The model under review builds one solid part; all positions refer to its coordinate system, in mm. Face numbers are marked on the shaded views. A direction names the side the tool comes from. Coordinates: 2 decimals unless noted, no trailing zeros. Order: outer loops, then holes, each group sorted by start corner. A loop starts at its lowest first (then second) coordinate and runs counter-clockwise, first axis right, second up. Notation, with made-up numbers: M 69.25,39 L 113.25,39 A32 ccw 113.25,71 Z; hole C 87.25,6 d5. An arc over 180 degrees is marked long. Answer in a Markdown table with one row per item.
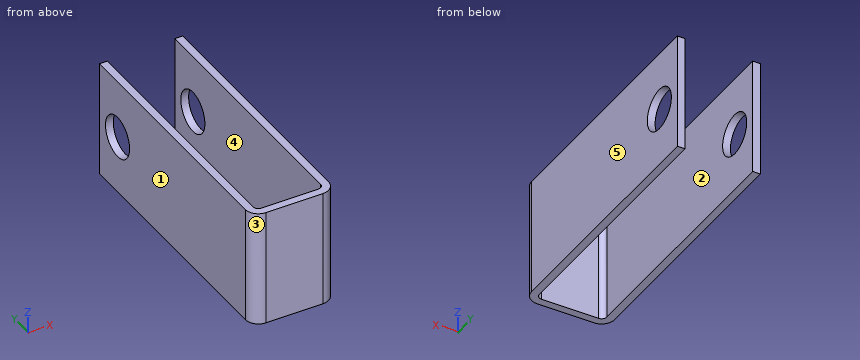
from build123d import *

# Parameters (mm, degrees)
BOSS_EXTRUDE1_DEPTH = 45
SKETCH2_R           = 8
CUT_EXTRUDE1_DEPTH  = 116.987068245


with BuildPart() as part:
    # Sketch1 → Boss-Extrude1 (new body)
    with BuildSketch(Plane.XY):
        with BuildLine():
            Line((0, 0), (0, -97))
            ThreePointArc((0, -97), (1.464466094, -100.535533906), (5, -102))
            Line((5, -102), (27, -102))
            ThreePointArc((27, -102), (30.535533906, -100.535533906), (32, -97))
            Line((32, -97), (32, 0))
            Line((32, 0), (29, 0))
            Line((29, 0), (29, -97))
            ThreePointArc((29, -97), (28.414213562, -98.414213562), (27, -99))
            Line((27, -99), (5, -99))
            ThreePointArc((5, -99), (3.585786438, -98.414213562), (3, -97))
            Line((3, -97), (3, 0))
            Line((3, 0), (0, 0))
        make_face()
    extrude(amount=BOSS_EXTRUDE1_DEPTH)

    # Sketch2 → Cut-Extrude1 (cut, through all)
    with BuildSketch(Plane(origin=(32, 0, 0), x_dir=(0, 0, -1), z_dir=(1, 0, 0))):
        with Locations((-22.5, -12)):
            Circle(SKETCH2_R)
    extrude(amount=-CUT_EXTRUDE1_DEPTH, mode=Mode.SUBTRACT)


solid = part.part
(1) Insertion check: P1, Ø10, axis at x = 11, z = 14.5, coming from the +Y side. The pin has a flat end and moves straight along its axis. Give the tip position at first contact, or say it passes through.
Report:
| item | result |
|---|---|
| P1 | y = -99 |
(2) Take a section at D-D (z = 6.5). Write out the cut boundary in (x, y).
Report:
| item | result |
|---|---|
| outline | M 0,-97 A5 ccw 5,-102 L 27,-102 A5 ccw 32,-97 L 32,0 L 29,0 L 29,-97 A2 cw 27,-99 L 5,-99 A2 cw 3,-97 L 3,0 L 0,0 Z |
(3) Take a section at B-B (y = -12). Write out the cut boundary in (x, z).
Report:
| item | result |
|---|---|
| outline | M 0,0 L 3,0 L 3,14.5 L 0,14.5 Z; M 0,30.5 L 3,30.5 L 3,45 L 0,45 Z; M 29,0 L 32,0 L 32,14.5 L 29,14.5 Z; M 29,30.5 L 32,30.5 L 32,45 L 29,45 Z |
(4) The part is to be moulded in two halves that separate along X. For the marked faces 3, 4 and 5, say which applies: +X half, -X half, draft (parallel to the pull), parting line (faces both ways), or undercut.
Report:
| item | result |
|---|---|
| face 3 | -X half |
| face 4 | undercut |
| face 5 | +X half |
(5) Take a section at C-C (y = -28). Write out the cut boundary in (x, z), then the cut area to 3 significant figures.
Report:
| item | result |
|---|---|
| outline | M 0,0 L 3,0 L 3,45 L 0,45 Z; M 29,0 L 32,0 L 32,45 L 29,45 Z |
| area | 270 mm^2 |
(6) Take a section at A-A (z = 22.5). Write out the cut boundary in (x, y), then the cut area to 3 significant figures.
Report:
| item | result |
|---|---|
| outline | M 0,-97 A5 ccw 5,-102 L 27,-102 A5 ccw 32,-97 L 32,-20 L 29,-20 L 29,-97 A2 cw 27,-99 L 5,-99 A2 cw 3,-97 L 3,-20 L 0,-20 Z; M 0,-4 L 3,-4 L 3,0 L 0,0 Z; M 29,-4 L 32,-4 L 32,0 L 29,0 Z |
| area | 585 mm^2 |
(7) To check wall thickness, follow line 1 (X direction, y = -47.5, z = 20.5); line 2 (Y direction, x = 18, z = 11.5); line 3 (Y direction, x = 1.1, z = 22.5). State the ranges of each line that lie inside material, in increasing order. Write a range as [from, to].
Report:
| item | result |
|---|---|
| line 1 | [0, 3], [29, 32] |
| line 2 | [-102, -99] |
| line 3 | [-100.13, -20], [-4, 0] |
(8) Machinability: for the marked faces 1 and 2, which of the approach directions +Z, -Z, +X, -X, +Y, -Y give a long, thin tool a straight path to every point of the face, cutting with its end or side? Answer none if there is none.
Report:
| item | result |
|---|---|
| face 1 | +Z, -Z, -X, +Y, -Y |
| face 2 | +Z, -Z, +Y |
